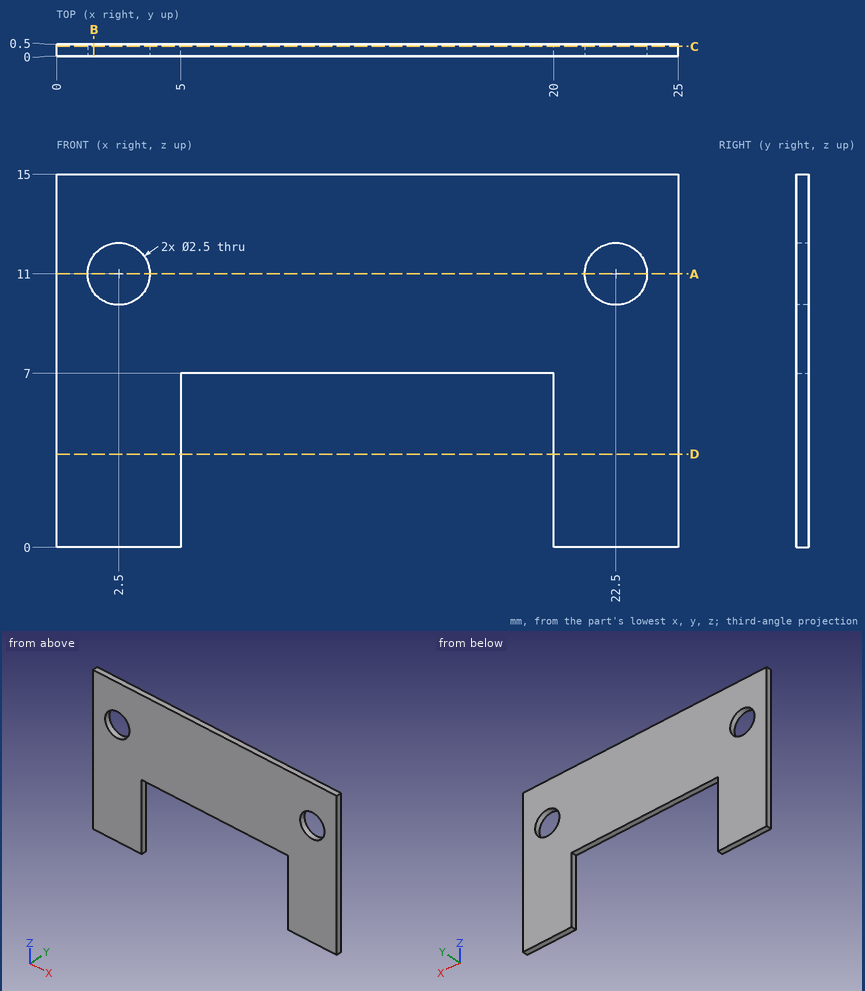
Job drawing, mm, ordinate dimensions from the low corner. One solid piece. Coordinates: 2 decimals unless noted, no trailing zeros. Write each loop counter-clockwise with the first axis right and the second up, starting at its lowest first coordinate (ties: lowest second). Pieces come first, ordered by that corner, then holes.
Item 1: Slice it at D-D (z = 3.75). Write the cut outline in (x, y), and give its area (3 significant figures).
Item 2: Pin check, flat tips, straight feed: pin 1 (3 mm diameter, centred on x = 2.5, z = 11, fed in from +Y); pin 2 (2 mm diameter, centred on x = 22.5, z = 11, fed in from -Y). Stop position of each tip, or through.
Item 3: Slice it at B-B (x = 1.5). Write the cut outline in (y, z), and give its area (3 significant figures).
Item 4: Slice it at C-C (y = 0.4). Write the cut outline in (x, z).
Item 5: Slice it at A-A (z = 11). Write the cut outline in (x, y).
Item 6: Probe line 1 (X direction, y = 0.3, z = 11); line 2 (X direction, y = 0.4, z = 6.75); line 3 (Z direction, x = 6.5, y = 0.3). List the from-to ranges inside material, lowest first.
Results found:
1. outline: (0, 0) - (5, 0) - (5, 0.5) - (0, 0.5) - close; (20, 0) - (25, 0) - (25, 0.5) - (20, 0.5) - close
1. area: 5.00 mm2
2. pin 1: stops at y = 0.5
2. pin 2: passes through
3. outline: (0, 0) - (0.5, 0) - (0.5, 10.25) - (0, 10.25) - close; (0, 11.75) - (0.5, 11.75) - (0.5, 15) - (0, 15) - close
3. area: 6.75 mm2
4. outline: (0, 0) - (5, 0) - (5, 7) - (20, 7) - (20, 0) - (25, 0) - (25, 15) - (0, 15) - close; hole circle Ø2.5 at (2.5, 11); hole circle Ø2.5 at (22.5, 11)
5. outline: (0, 0) - (1.25, 0) - (1.25, 0.5) - (0, 0.5) - close; (3.75, 0) - (21.25, 0) - (21.25, 0.5) - (3.75, 0.5) - close; (23.75, 0) - (25, 0) - (25, 0.5) - (23.75, 0.5) - close
6. line 1: x = 0 to 1.25, 3.75 to 21.25, 23.75 to 25
6. line 2: x = 0 to 5, 20 to 25
6. line 3: z = 7 to 15
